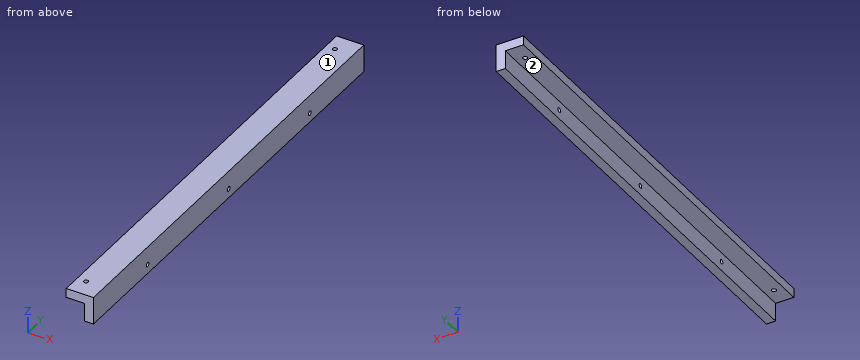
```python
from build123d import *

# Parameters (mm, degrees)
BOSS_EXTRUDE1_DEPTH = 250
SKETCH3_R           = 1.2
CUT_EXTRUDE1_DEPTH  = 10
SKETCH4_R           = 1.2
CUT_EXTRUDE2_DEPTH  = 5


with BuildPart() as part:
    # Sketch1 → Boss-Extrude1 (new body)
    with BuildSketch(Plane(origin=(0, 0, 0), x_dir=(1, 0, 0), z_dir=(0, 1, 0))):
        Polygon((0, 0), (15, 0), (15, 15), (10, 15), (10, 5), (0, 5), align=None)
    extrude(amount=BOSS_EXTRUDE1_DEPTH)

    # Sketch3 → Cut-Extrude1 (cut)
    with BuildSketch(Plane.ZY.offset(-10)):
        with Locations((-10, 50)):
            Circle(SKETCH3_R)
        with Locations((-10, 125)):
            Circle(SKETCH3_R)
        with Locations((-10, 200)):
            Circle(SKETCH3_R)
    extrude(amount=-CUT_EXTRUDE1_DEPTH, mode=Mode.SUBTRACT)

    # Sketch4 → Cut-Extrude2 (cut)
    with BuildSketch(Plane.XY):
        with Locations((5, 10)):
            Circle(SKETCH4_R)
        with Locations((5, 240)):
            Circle(SKETCH4_R)
    extrude(amount=-CUT_EXTRUDE2_DEPTH, mode=Mode.SUBTRACT)


solid = part.part
```
Check sheet for the modelled part. Datum: model origin and axes. Units: mm. Face numbers are marked on the shaded views. A direction names the side the tool comes from. Round coordinates to 2 decimals unless told otherwise and drop trailing zeros. Order: outer loops, then holes, each group sorted by start corner. A loop starts at its lowest first (then second) coordinate and runs counter-clockwise, first axis right, second up. Notation, with made-up numbers: (29.5, 62) - (66.5, 62) arc R25 ccw to (66.5, 90) - close; hole circle Ø2 at (15.5, -23). An arc over 180 degrees is marked (long way). Write item = value, one per line.
Q1. Thickness scan on line 1 along Y through (x, z) = (5, -1.3); line 2 along Y through (x, z) = (11.4, -10); line 3 along Z through (x, y) = (13.05, 200). Record the ranges inside material, lowest first.
Computed:
line_1 = 0 to 8.8, 11.2 to 238.8, 241.2 to 250
line_2 = 0 to 48.8, 51.2 to 123.8, 126.2 to 198.8, 201.2 to 250
line_3 = -15 to -11.2, -8.8 to 0
Q2. Go/stop test with flat-tipped pins: pin 1 (2 mm diameter, centred on x = 3, y = 86.5, fed in from +Z); pin 2 (3 mm diameter, centred on y = 118.5, z = -8, fed in from -X); pin 3 (1.9 mm diameter, centred on y = 200, z = -10, fed in from -X); pin 4 (4 mm diameter, centred on x = 5, y = 10, fed in from -Z). Record where each tip stops, or that it passes through.
Computed:
pin_1 = 0
pin_2 = 10
pin_3 = through
pin_4 = -5
Q3. Tool access check on the marked faces 1 and 2. Record the directions out of +Z, -Z, +X, -X, +Y, -Y that give a thin tool (end or side, any length) a straight path to the whole face; none if there is none.
Computed:
face_1 = +Z, +X, -X, +Y, -Y
face_2 = -Z, -X, +Y, -Y
Q4. Section check A-A (y = 137.5). Record the boundary of the cut face in (x, z), and give its area (3 significant figures).
Computed:
outline = (0, -5) - (10, -5) - (10, -15) - (15, -15) - (15, 0) - (0, 0) - close
area = 125 mm^2
